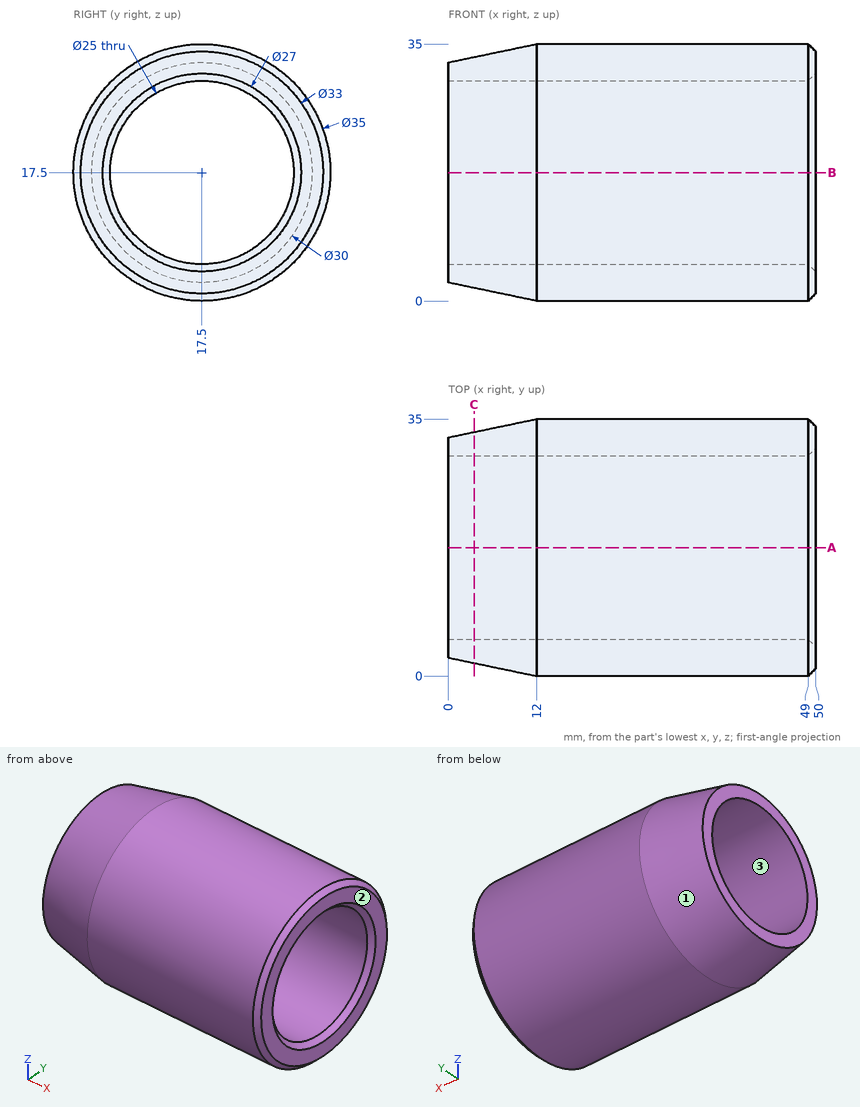
Geometry check sheet. Reference: drawing and pictorial views, mm from the part's lowest x, y, z. Give positions to 0.01 mm unless a question says otherwise; leave off trailing zeros. Write each loop counter-clockwise with the first axis right and the second up, starting at its lowest first coordinate (ties: lowest second). Pieces come first, ordered by that corner, then holes.
Item 1: Cross-section at A-A (y = 17.5). Enter the section's corners in (x, z).
Item 2: Cross-section at C-C (x = 3.5). Enter the section's corners in (y, z).
Item 3: Gauge pin test, flat ends, axial feed: pin 1 (5 mm diameter, centred on x = 28.5, y = 27, fed in from +Z); pin 2 (1.5 mm diameter, centred on x = 27.5, z = 24.5, fed in from -Y); pin 3 (5 mm diameter, centred on x = 32, z = 14.5, fed in from -Y). Record the tip position at first contact, or that the pin passes through.
Item 4: Draft check along Z on the marked faces 1, 2 and 3. Enter one of: released by +Z, released by -Z, zero draft, split by the parting line, or undercut.
Item 5: Scan lines: L1, parallel to Z at x = 13, y = 17; L2, parallel to Y at x = 25.5, z = 17.5; L3, parallel to Y at x = 18.5, z = 19. Record each from-to range of solid material in increasing order.
Report:
1. outline: (0, 2.5) - (12, 0) - (49, 0) - (50, 1) - (50, 4) - (49, 5) - (0, 5) - close; (0, 30) - (49, 30) - (50, 31) - (50, 34) - (49, 35) - (12, 35) - (0, 32.5) - close
2. outline: circle Ø31.46 at (17.5, 17.5); hole circle Ø25 at (17.5, 17.5)
3. pin 1: stops at z = 33.54
3. pin 2: stops at y = 1.15
3. pin 3: stops at y = 0.01
4. face 1: split by the parting line
4. face 2: zero draft
4. face 3: undercut
5. L1: z = 0.01 to 5.01, 29.99 to 34.99
5. L2: y = 0 to 5, 30 to 35
5. L3: y = 0.06 to 5.09, 29.91 to 34.94
